```python
from build123d import *

# Parameters (mm, degrees)
SKETCH_1_R      = 3
EXTRUDE_1_DEPTH = 12
SKETCH_2_R      = 6
EXTRUDE_2_DEPTH = 4
CHAMFER_1_SIZE  = 1
EXTRUDE_START   = 4
SKETCH_3_R      = 6
EXTRUDE_3_DEPTH = 4
CHAMFER_2_SIZE  = 1


with BuildPart() as part:
    # 草图1 → 凸台-拉伸1 (new body)
    with BuildSketch(Plane.XY):
        Circle(SKETCH_1_R)
    extrude(amount=EXTRUDE_1_DEPTH)

    # 草图2 → 凸台-拉伸2 (add)
    with BuildSketch(Plane.XY.offset(12)):
        Circle(SKETCH_2_R)
    extrude(amount=EXTRUDE_2_DEPTH)

    # 倒角1
    chamfer_1_edges = [part.edges().sort_by_distance(p)[0] for p in [
        (-6, 0, 16),
    ]]
    chamfer(chamfer_1_edges, length=CHAMFER_1_SIZE)

    # 草图3 → 凸台-拉伸3 (add)
    with BuildSketch(Plane(origin=(0, 0, 0), x_dir=(-1, 0, 0), z_dir=(0, 0, -1)).offset(EXTRUDE_START)):
        with Locations(Location((0, 0, 0), (0, 0, 180))):
            Circle(SKETCH_3_R)
    extrude(amount=-EXTRUDE_3_DEPTH)

    # 倒角2
    chamfer_2_edges = [part.edges().sort_by_distance(p)[0] for p in [
        (-6, 0, -4),
    ]]
    chamfer(chamfer_2_edges, length=CHAMFER_2_SIZE)


solid = part.part
```
Verification items for the finished model (mm, model axes). A direction names the side the tool comes from. Round coordinates to 2 decimals unless told otherwise and drop trailing zeros. Write each loop counter-clockwise with the first axis right and the second up, starting at its lowest first coordinate (ties: lowest second). Pieces come first, ordered by that corner, then holes.
1. Scan lines: L1, parallel to Z at x = -2.5, y = -4.25; L2, parallel to Y at x = -0.25, z = 13.25; L3, parallel to Y at x = 0, z = 0.5. Record each from-to range of solid material in increasing order.
2. Access from +Z, -Z, +X, -X, +Y, -Y to the whole of each face (thin tool, end or side, straight path). Record for faces 4 (the flat face through (0, 0, -4)), 5 (the cylindrical face through (-3, 0, 6)).
3. Gauge pin test, flat ends, axial feed: P1, Ø3, axis at x = -3.5, z = 4, coming from the -Y side; P2, Ø3, axis at x = 4, z = -1.5, coming from the -Y side; P3, Ø2, axis at y = -3, z = 4.5, coming from the +X side. Record the tip position at first contact, or that the pin passes through.
4. Section check D-D on z = 0.5. Enter the section's corners in (x, y), plus the area to 3 significant figures.
5. Section check C-C on z = -1.5. Enter the section's corners in (x, y), plus the area to 3 significant figures.
6. Section check A-A on y = 0. Enter the section's corners in (x, z), plus the area to 3 significant figures.
7. Draft check along Z on faces 1 (the flat face through (-3, 1, 0)), 2 (the flat face through (0, 0, 16)), 3 (the cylindrical face through (-6, 0, 13)). Enter one of: +Z half, -Z half, draft (parallel to the pull), parting line (faces both ways), or undercut.
Answer:
1. L1: z = -4 to 0, 12 to 16
1. L2: y = -5.99 to 5.99
1. L3: y = -3 to 3
2. face 4: -Z, +X, -X, +Y, -Y
2. face 5: none
3. P1: stops at y = -2.24
3. P2: stops at y = -5.45
3. P3: stops at x = 2.24
4. outline: circle Ø6 at (0, 0)
4. area: 28.3 mm2
5. outline: circle Ø12 at (0, 0)
5. area: 113 mm2
6. outline: (-6, -3) - (-5, -4) - (5, -4) - (6, -3) - (6, 0) - (3, 0) - (3, 12) - (6, 12) - (6, 15) - (5, 16) - (-5, 16) - (-6, 15) - (-6, 12) - (-3, 12) - (-3, 0) - (-6, 0) - close
6. area: 166 mm2
7. face 1: undercut
7. face 2: +Z half
7. face 3: draft
